from build123d import *

# Parameters (mm, degrees)
EXTRUDE_1_DEPTH     = 16
SKETCH_2_W          = 30
SKETCH_2_H          = 20
SKETCH_2_W_2        = 23
SKETCH_2_H_2        = 35
CUT_EXTRUDE_1_DEPTH = 3
CUT_EXTRUDE_2_DEPTH = 5
CUT_EXTRUDE_3_REACH = 80.481
SKETCH_4_R          = 2.75
CUT_EXTRUDE_4_REACH = 79.925
SKETCH_5_R          = 2.75
SKETCH_6_R          = 5
CUT_EXTRUDE_5_DEPTH = 9
SKETCH_7_R          = 2.1
CUT_EXTRUDE_6_DEPTH = 12.5
SKETCH_8_R          = 2.5
CUT_EXTRUDE_7_DEPTH = 10


with BuildPart() as part:
    # 草图1 → 凸台-拉伸1 (new body)
    with BuildSketch(Plane.XY):
        Polygon((-47.83180778, 24.741418764), (64.16819222, 24.741418764), (64.16819222, 4.741418764), (19.66819222, 4.741418764), (19.66819222, -42.258581236), (-3.33180778, -42.258581236), (-3.33180778, 4.741418764), (-47.83180778, 4.741418764), align=None)
    extrude(amount=EXTRUDE_1_DEPTH)

    # 草图2 → 切除-拉伸1 (cut)
    with BuildSketch(Plane(origin=(0, 0, 0), x_dir=(-1, 0, 0), z_dir=(0, 0, -1))):
        with Locations((-49.16819222, 14.741418764)):
            Rectangle(SKETCH_2_W, SKETCH_2_H)
        with Locations((-8.16819222, -24.758581236)):
            Rectangle(SKETCH_2_W_2, SKETCH_2_H_2)
        with Locations((32.83180778, 14.741418764)):
            Rectangle(SKETCH_2_W, SKETCH_2_H)
    extrude(amount=-CUT_EXTRUDE_1_DEPTH, mode=Mode.SUBTRACT)

    # 草图3 → 切除-拉伸2 (cut)
    with BuildSketch(Plane.XY.offset(16)):
        with BuildLine():
            Line((10.66819222, 24.741418764), (5.66819222, 24.741418764))
            Line((5.66819222, 24.741418764), (5.66819222, -6.755194133))
            ThreePointArc((5.66819222, -6.755194133), (6.253978657, -8.169407696), (7.66819222, -8.755194133))
            Line((7.66819222, -8.755194133), (8.66819222, -8.755194133))
            ThreePointArc((8.66819222, -8.755194133), (10.082405782, -8.169407696), (10.66819222, -6.755194133))
            Line((10.66819222, -6.755194133), (10.66819222, 24.741418764))
        make_face()
    extrude(amount=-CUT_EXTRUDE_2_DEPTH, mode=Mode.SUBTRACT)

    # 草图4 → 切除-拉伸3 (cut, up to next)
    with BuildSketch(Plane.XY.offset(16), mode=Mode.PRIVATE) as cut_extrude_3_sk1:
        with Locations((56.16819222, 14.741418764)):
            Circle(SKETCH_4_R)
    cut_extrude_3_tool1 = extrude(cut_extrude_3_sk1.sketch, amount=-CUT_EXTRUDE_3_REACH, mode=Mode.PRIVATE) & part.part
    # 草图4 → 切除-拉伸3 (cut, up to next)
    with BuildSketch(Plane.XY.offset(16), mode=Mode.PRIVATE) as cut_extrude_3_sk2:
        with Locations((42.43519222, 14.741418764)):
            Circle(SKETCH_4_R)
    cut_extrude_3_tool2 = extrude(cut_extrude_3_sk2.sketch, amount=-CUT_EXTRUDE_3_REACH, mode=Mode.PRIVATE) & part.part
    # 草图4 → 切除-拉伸3 (cut, up to next)
    with BuildSketch(Plane.XY.offset(16), mode=Mode.PRIVATE) as cut_extrude_3_sk3:
        with Locations((-26.68180778, 14.741418764)):
            Circle(SKETCH_4_R)
    cut_extrude_3_tool3 = extrude(cut_extrude_3_sk3.sketch, amount=-CUT_EXTRUDE_3_REACH, mode=Mode.PRIVATE) & part.part
    # 草图4 → 切除-拉伸3 (cut, up to next)
    with BuildSketch(Plane.XY.offset(16), mode=Mode.PRIVATE) as cut_extrude_3_sk4:
        with Locations((-40.41480778, 14.741418764)):
            Circle(SKETCH_4_R)
    cut_extrude_3_tool4 = extrude(cut_extrude_3_sk4.sketch, amount=-CUT_EXTRUDE_3_REACH, mode=Mode.PRIVATE) & part.part
    add(cut_extrude_3_tool1.solids().sort_by_distance((56.168192, 14.741419, 16))[0], mode=Mode.SUBTRACT)
    add(cut_extrude_3_tool2.solids().sort_by_distance((42.435192, 14.741419, 16))[0], mode=Mode.SUBTRACT)
    add(cut_extrude_3_tool3.solids().sort_by_distance((-26.681808, 14.741419, 16))[0], mode=Mode.SUBTRACT)
    add(cut_extrude_3_tool4.solids().sort_by_distance((-40.414808, 14.741419, 16))[0], mode=Mode.SUBTRACT)

    # 草图5 → 切除-拉伸4 (cut, up to next)
    with BuildSketch(Plane(origin=(0, 0, 3), x_dir=(-1, 0, 0), z_dir=(0, 0, -1)), mode=Mode.PRIVATE) as cut_extrude_4_sk1:
        with Locations((-8.16819222, -15.258581236)):
            Circle(SKETCH_5_R)
    cut_extrude_4_tool1 = extrude(cut_extrude_4_sk1.sketch, amount=-CUT_EXTRUDE_4_REACH, mode=Mode.PRIVATE) & part.part
    # 草图5 → 切除-拉伸4 (cut, up to next)
    with BuildSketch(Plane(origin=(0, 0, 3), x_dir=(-1, 0, 0), z_dir=(0, 0, -1)), mode=Mode.PRIVATE) as cut_extrude_4_sk2:
        with Locations((-8.16819222, -34.258581236)):
            Circle(SKETCH_5_R)
    cut_extrude_4_tool2 = extrude(cut_extrude_4_sk2.sketch, amount=-CUT_EXTRUDE_4_REACH, mode=Mode.PRIVATE) & part.part
    add(cut_extrude_4_tool1.solids().sort_by_distance((8.168192, -15.258581, 3))[0], mode=Mode.SUBTRACT)
    add(cut_extrude_4_tool2.solids().sort_by_distance((8.168192, -34.258581, 3))[0], mode=Mode.SUBTRACT)

    # 草图6 → 切除-拉伸5 (cut)
    with BuildSketch(Plane.XY.offset(16)):
        with Locations((-40.41480778, 14.741418764)):
            Circle(SKETCH_6_R)
        with Locations((-26.68180778, 14.741418764)):
            Circle(SKETCH_6_R)
        with Locations((42.43519222, 14.741418764)):
            Circle(SKETCH_6_R)
        with Locations((56.16819222, 14.741418764)):
            Circle(SKETCH_6_R)
        with Locations((8.16819222, -15.258581236)):
            Circle(SKETCH_6_R)
        with Locations((8.16819222, -34.258581236)):
            Circle(SKETCH_6_R)
    extrude(amount=-CUT_EXTRUDE_5_DEPTH, mode=Mode.SUBTRACT)

    # 草图7 → 切除-拉伸6 (cut)
    with BuildSketch(Plane.XY.offset(16)):
        with Locations((25.66819222, 14.741418764)):
            Circle(SKETCH_7_R)
        with Locations(Location((-9.33180778, 14.741418764, 0), (0, 0, 180))):
            Circle(SKETCH_7_R)
        with Locations((8.16819222, -24.258581236)):
            Circle(SKETCH_7_R)
    extrude(amount=-CUT_EXTRUDE_6_DEPTH, mode=Mode.SUBTRACT)

    # 草图8 → 切除-拉伸7 (cut)
    with BuildSketch(Plane.XY.offset(16)):
        with Locations((-9.33180778, 14.741418764)):
            Circle(SKETCH_8_R)
        with Locations((25.66819222, 14.741418764)):
            Circle(SKETCH_8_R)
        with Locations((8.16819222, -24.258581236)):
            Circle(SKETCH_8_R)
    extrude(amount=-CUT_EXTRUDE_7_DEPTH, mode=Mode.SUBTRACT)


solid = part.part
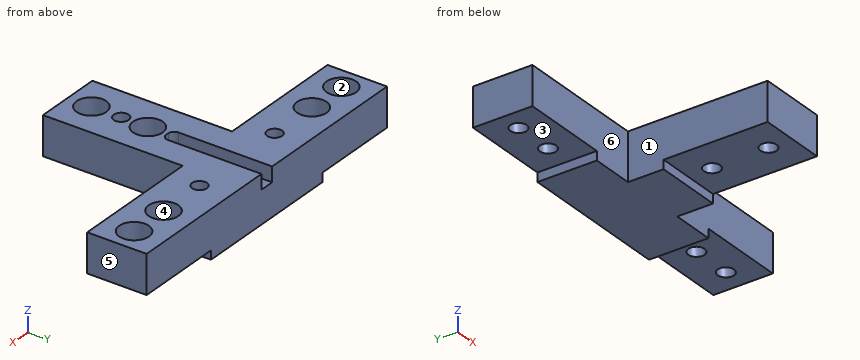
Source: CAD feature listing. Evaluate the final solid. Frame: model axes, mm. Face numbers are marked on the shaded views. A direction names the side the tool comes from. Coordinates: 2 decimals unless noted, no trailing zeros. Write each loop counter-clockwise with the first axis right and the second up, starting at its lowest first coordinate (ties: lowest second). Pieces come first, ordered by that corner, then holes. Notation, with made-up numbers: M 20.25,-26 L 53.25,-26 A23 ccw 53.25,1 Z; hole C 81.25,84.5 d9. An arc over 180 degrees is marked long. Use a Markdown table: item, result.
1) First-contact query: pin 1 Ø4.5 at (x, y) = (25.67, 14.74) entering from +Z; pin 2 Ø6 at (y, z) = (-6, 10) entering from -X; pin 3 Ø22 at (x, y) = (49, 19.5) entering from -Z. Flat tips, straight axial feed; report the tip coordinate or a pass-through.
Conclusion:
| item | result |
|---|---|
| pin 1 | stops at z = 6 |
| pin 2 | stops at x = -3.33 |
| pin 3 | stops at z = 3 |
2) Mould query, pull axis Y, two halves, no side actions, for the marked faces 4, 5 and 6. Classes: pulls with the +Y half, pulls with the -Y half, needs draft (parallel to the pull), parting line crosses it, or undercut.
Conclusion:
| item | result |
|---|---|
| face 4 | undercut |
| face 5 | needs draft |
| face 6 | pulls with the -Y half |
3) Ray query, L1, parallel to X at y = -24, z = 8; L2, parallel to X at y = 19, z = 11.25; L3, parallel to Z at x = -30.5, y = 20. Return the intervals inside material, ascending.
Conclusion:
| item | result |
|---|---|
| L1 | x = -3.33 to 5.68, 10.65 to 19.67 |
| L2 | x = -47.83 to -43.03, -37.79 to -29.3, -24.06 to 5.67, 10.67 to 39.82, 45.06 to 53.55, 58.79 to 64.17 |
| L3 | z = 3 to 16 |
4) Section A-A, the plane x = -39.5. Output: boundary loops of the cut face in (y, z), then the cut area to 3 significant figures.
Conclusion:
| item | result |
|---|---|
| outline | M 4.74,3 L 12.15,3 L 12.15,7 L 9.83,7 L 9.83,16 L 4.74,16 Z; M 17.33,3 L 24.74,3 L 24.74,16 L 19.66,16 L 19.66,7 L 17.33,7 Z |
| area | 151 mm^2 |
5) Section C-C, the plane y = 7. Output: boundary loops of the cut face in (x, z), then the cut area to 3 significant figures.
Conclusion:
| item | result |
|---|---|
| outline | M -47.83,3 L -17.83,3 L -17.83,0 L 34.17,0 L 34.17,3 L 64.17,3 L 64.17,16 L 10.67,16 L 10.67,11 L 5.67,11 L 5.67,16 L -47.83,16 Z |
| area | 1,590 mm^2 |
6) Reachability of the marked faces 1, 2 and 3 from +Z, -Z, +X, -X, +Y, -Y: full face, straight path, thin tool, end or side. Return the list, or none.
Conclusion:
| item | result |
|---|---|
| face 1 | +Z, -Z, -X, -Y |
| face 2 | +Z |
| face 3 | -Z, -X, +Y, -Y |
7) Section D-D, the plane x = 35.5. Output: boundary loops of the cut face in (y, z), then the cut area to 3 significant figures.
Conclusion:
| item | result |
|---|---|
| outline | M 4.74,3 L 24.74,3 L 24.74,16 L 4.74,16 Z |
| area | 260 mm^2 |
8) Section B-B, the plane z = 8.5. Give the number of separate pieces and of enclosed holes in the cut face, then the cut area to 3 significant figures.
Conclusion:
| item | result |
|---|---|
| separate pieces | 1 |
| enclosed holes | 9 |
| area | 2,790 mm^2 |
